Could you check a few things on this model? Use its own coordinates, in mm. Face numbers are marked on the shaded views. A direction names the side the tool comes from. Give positions to 0.01 mm unless a question says otherwise; leave off trailing zeros. Order: outer loops, then holes, each group sorted by start corner. A loop starts at its lowest first (then second) coordinate and runs counter-clockwise, first axis right, second up. Notation, with made-up numbers: M 1,83.5 L 43,83.5 A31 ccw 43,113.5 Z; hole C 29.25,37.25 d9. An arc over 180 degrees is marked long. Use a Markdown table: item, result. Add a question column.
```python
from build123d import *

# Parameters (mm, degrees)
SKETCH1_W           = 40
SKETCH1_H           = 12
SKETCH1_R           = 2.25
SKETCH1_R_2         = 3
BOSS_EXTRUDE1_DEPTH = 3
SKETCH2_W           = 4
SKETCH2_H           = 12
BOSS_EXTRUDE2_DEPTH = 10
FILLET1_R           = 2


with BuildPart() as part:
    # Sketch1 → Boss-Extrude1 (new body)
    with BuildSketch(Plane.XY):
        with Locations((20, 6)):
            Rectangle(SKETCH1_W, SKETCH1_H)
        with Locations((20, 6)):
            Circle(SKETCH1_R, mode=Mode.SUBTRACT)
        with Locations((6, 6)):
            Circle(SKETCH1_R_2, mode=Mode.SUBTRACT)
    extrude(amount=BOSS_EXTRUDE1_DEPTH)

    # Sketch2 → Boss-Extrude2 (add)
    with BuildSketch(Plane.XY.offset(3)):
        with Locations((38, 6)):
            Rectangle(SKETCH2_W, SKETCH2_H)
    extrude(amount=BOSS_EXTRUDE2_DEPTH)

    # Fillet1
    fillet1_edges = [part.edges().sort_by_distance(p)[0] for p in [
        (36, 6, 3),
    ]]
    fillet(fillet1_edges, radius=FILLET1_R)


solid = part.part
```
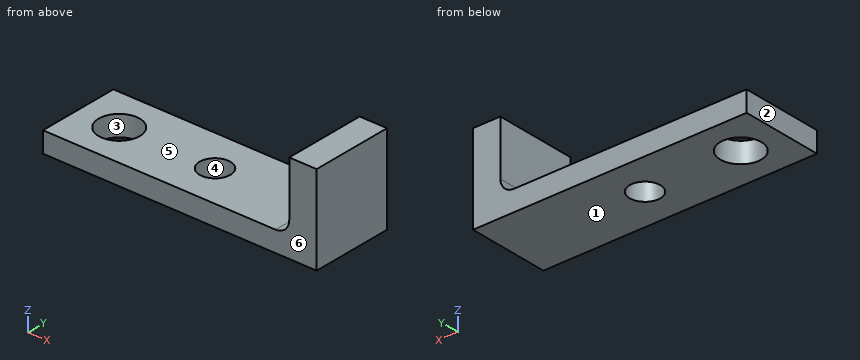
1) Suppose I cut it at B-B on y = 6. Please give me the cut outline in (x, z), and give its area (3 significant figures).
2) For pin 1 (3.5 mm diameter, centred on x = 6, y = 6, fed in from -Z); pin 2 (1.5 mm diameter, centred on y = 4.5, z = 7.5, fed in from -X); pin 3 (6 mm diameter, centred on x = 8, y = 6.5, fed in from +Z), each with a flat end and sliding along its axis, tell me the tip position at first contact or that it passes through.
3) We'd pull the mould along X, two halves only. Please class the marked faces 1, 2, 3 and 4: pulls with the +X half, pulls with the -X half, needs draft (parallel to the pull), parting line crosses it, or undercut.
4) Suppose I cut it at D-D on y = 1. Please give me the cut outline in (x, z), and give its area (3 significant figures).
5) Suppose I cut it at C-C on z = 2. Please give me the cut outline in (x, y).
6) For the marked faces 5 and 6, which set-ups out of +Z, -Z, +X, -X, +Y, -Y let a thin tool reach every point of the face, with its end or its side?
7) Please list where these lines run through material, in increasing order: line 1 (Y direction, x = 20, z = 0.75); line 2 (Y direction, x = 6, z = 1.9); line 3 (X direction, y = 7, z = 2). Write a range as from..to.
8) Suppose I cut it at A-A on x = 20. Please give me the cut outline in (y, z), and give its area (3 significant figures).
Values found:
| question | item | result |
|---|---|---|
| 1 | outline | M 0,0 L 3,0 L 3,3 L 0,3 Z; M 9,0 L 17.75,0 L 17.75,3 L 9,3 Z; M 22.25,0 L 40,0 L 40,13 L 36,13 L 36,5 A2 cw 34,3 L 22.25,3 Z |
| 1 | area | 129 mm^2 |
| 2 | pin 1 | passes through |
| 2 | pin 2 | stops at x = 36 |
| 2 | pin 3 | stops at z = 3 |
| 3 | face 1 | needs draft |
| 3 | face 2 | pulls with the -X half |
| 3 | face 3 | undercut |
| 3 | face 4 | undercut |
| 4 | outline | M 0,0 L 40,0 L 40,13 L 36,13 L 36,5 A2 cw 34,3 L 0,3 Z |
| 4 | area | 161 mm^2 |
| 5 | outline | M 0,0 L 40,0 L 40,12 L 0,12 Z; hole C 6,6 d6; hole C 20,6 d4.5 |
| 6 | face 5 | +Z, -X, +Y, -Y |
| 6 | face 6 | +Z, -Z, +X, -X, -Y |
| 7 | line 1 | y = 0..3.75, 8.25..12 |
| 7 | line 2 | y = 0..3, 9..12 |
| 7 | line 3 | x = 0..3.17, 8.83..17.98, 22.02..40 |
| 8 | outline | M 0,0 L 3.75,0 L 3.75,3 L 0,3 Z; M 8.25,0 L 12,0 L 12,3 L 8.25,3 Z |
| 8 | area | 22.5 mm^2 |
